Answer from the drawing. Dimensions are ordinates in mm from the lowest x, y and z of the part. Coordinates: 2 decimals unless noted, no trailing zeros. Write each loop counter-clockwise with the first axis right and the second up, starting at its lowest first coordinate (ties: lowest second). Pieces come first, ordered by that corner, then holes.
(1) Section B-B on x = 50 is taken. Write down the section's boundary in (y, z), then the cut area to 3 significant figures.
(2) Section A-A on y = 30 is taken. Write down the section's boundary in (x, z), then the cut area to 3 significant figures.
(3) Given pin 1 (8 mm diameter, centred on x = 50, y = 30, fed in from -Z), flat-ended and moving along its own axis, determine where the tip first touches the part or whether it passes through.
(4) Find the intervals of material crossed by probe 1 along Y at (x, z) = (130, 4); probe 2 along X at (y, z) = (26, 2.5); probe 3 along X at (y, z) = (31.5, 3.5), in increasing order.
(5) Section C-C on z = 3 is taken. Write down the section's boundary in (x, y), then the cut area to 3 significant figures.
(6) Section D-D on x = 125 is taken. Write down the section's boundary in (y, z).
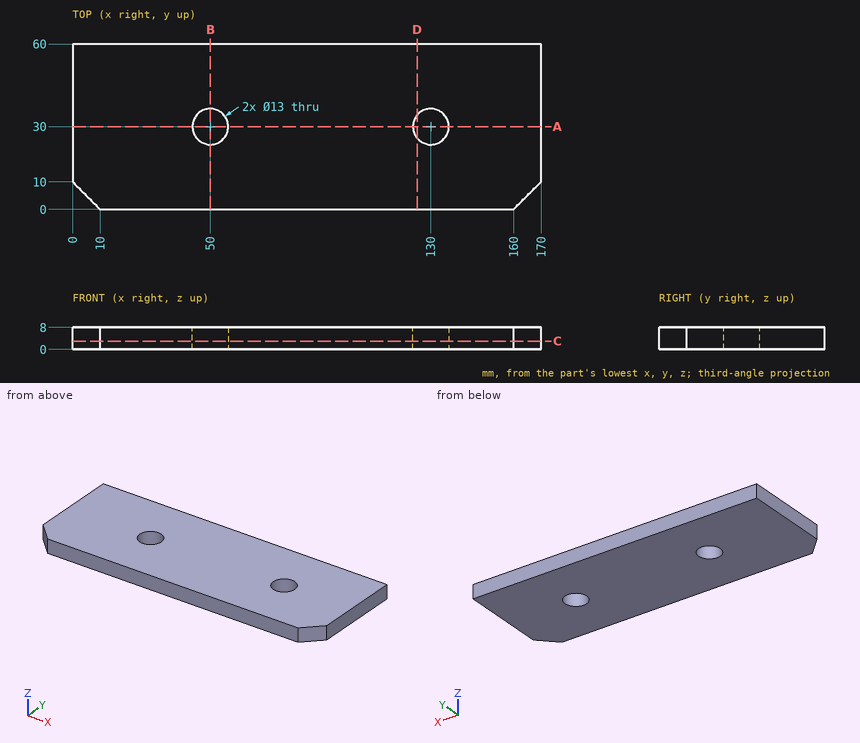
Response:
1. outline: (0, 0) - (23.5, 0) - (23.5, 8) - (0, 8) - close; (36.5, 0) - (60, 0) - (60, 8) - (36.5, 8) - close
1. area: 376 mm2
2. outline: (0, 0) - (43.5, 0) - (43.5, 8) - (0, 8) - close; (56.5, 0) - (123.5, 0) - (123.5, 8) - (56.5, 8) - close; (136.5, 0) - (170, 0) - (170, 8) - (136.5, 8) - close
2. area: 1,150 mm2
3. pin 1: passes through
4. probe 1: y = 0 to 23.5, 36.5 to 60
4. probe 2: x = 0 to 44.88, 55.12 to 124.88, 135.12 to 170
4. probe 3: x = 0 to 43.68, 56.32 to 123.68, 136.32 to 170
5. outline: (0, 10) - (10, 0) - (160, 0) - (170, 10) - (170, 60) - (0, 60) - close; hole circle Ø13 at (50, 30); hole circle Ø13 at (130, 30)
5. area: 9,830 mm2
6. outline: (0, 0) - (25.85, 0) - (25.85, 8) - (0, 8) - close; (34.15, 0) - (60, 0) - (60, 8) - (34.15, 8) - close
